Geometry check sheet. Reference: the model listing, model coordinates, mm. Face numbers are marked on the shaded views. Coordinates: 2 decimals unless noted, no trailing zeros. Loops run counter-clockwise (first coordinate to the right, second up) from the corner with the lowest first, then second, coordinate; pieces in that order, holes last. Notation, with made-up numbers: (86.25, 14.5) - (123.25, 14.5) arc R31 ccw to (123.25, 50.5) - close; hole circle Ø10 at (2, 59). An arc over 180 degrees is marked (long way). One line per item, written item: value.
from build123d import *

# Parameters (mm, degrees)
SKETCH_1_R      = 18
EXTRUDE_1_DEPTH = 12


with BuildPart() as part:
    # 草图1 → 凸台-拉伸1 (new body)
    with BuildSketch(Plane.XY):
        Polygon((24, 0), (12, 20.784609691), (-12, 20.784609691), (-24, 0), (-12, -20.784609691), (12, -20.784609691), align=None)
        Circle(SKETCH_1_R, mode=Mode.SUBTRACT)
    extrude(amount=EXTRUDE_1_DEPTH)

    # 草图2 → 切除-旋转1 (revolve, cut)
    with BuildSketch(Plane(origin=(0, 0, 0), x_dir=(1, 0, 0), z_dir=(0, 1, 0))):
        Polygon((-24, 0), (-24, -2.309401077), (-20, 0), align=None)
        Polygon((-24, -12), (-24, -9.690598923), (-20, -12), align=None)
    revolve(axis=Axis((0, 0, -5.971832554), (0, 0, 1)), mode=Mode.SUBTRACT)


solid = part.part
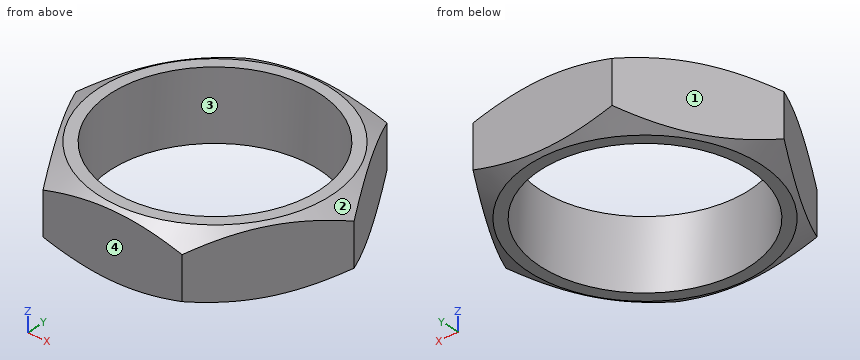
(1) Release check for a two-part mould opening along Y. For the marked faces 1, 2, 3 and 4 record: pulls with the +Y half, pulls with the -Y half, needs draft (parallel to the pull), parting line crosses it, or undercut.
Reply:
face 1: pulls with the +Y half
face 2: parting line crosses it
face 3: undercut
face 4: pulls with the -Y half
(2) Cross-section at A-A on z = 4. Record the cut outline in (x, y).
Reply:
outline: (-24, 0) - (-12, -20.78) - (12, -20.78) - (24, 0) - (12, 20.78) - (-12, 20.78) - close; hole circle Ø36 at (0, 0)
(3) Cross-section at B-B on x = 0. Record the cut outline in (y, z), and give its area (3 significant figures).
Reply:
outline: (-20.78, 0.45) - (-20, 0) - (-18, 0) - (-18, 12) - (-20, 12) - (-20.78, 11.55) - close; (18, 0) - (20, 0) - (20.78, 0.45) - (20.78, 11.55) - (20, 12) - (18, 12) - close
area: 66.1 mm2
(4) Material ranges on probe 1 along Y at (x, z) = (0, 3); probe 2 along X at (y, z) = (16, 2.75); probe 3 along X at (y, z) = (-9.5, 8.5), recorded low to high. Write a range as from..to.
Reply:
probe 1: -20.78..-18, 18..20.78
probe 2: -14.76..-8.25, 8.25..14.76
probe 3: -18.52..-15.29, 15.29..18.52
(5) Go/stop test with flat-tipped pins: pin 1 Ø6 at (y, z) = (-4, 7) entering from -X; pin 2 Ø2 at (x, z) = (14.5, 8.5) entering from -Y; pin 3 Ø3 at (y, z) = (2, 4.5) entering from +X; pin 4 Ø4 at (x, y) = (4, -14) entering from -Z. Record where each tip stops, or that it passes through.
Reply:
pin 1: x = -23.42
pin 2: y = -18.19
pin 3: x = 23.71
pin 4: through
